Geometry: final body of the model. Coordinates: model frame, mm. A direction names the side the tool comes from. Round coordinates to 2 decimals unless told otherwise and drop trailing zeros. Write each loop counter-clockwise with the first axis right and the second up, starting at its lowest first coordinate (ties: lowest second). Pieces come first, ordered by that corner, then holes. Notation, with made-up numbers: (-40, 81.25) -> (7, 81.25) arc R22 ccw to (7, 88.25) -> close; hole circle Ø8 at (83, -39). An arc over 180 degrees is marked (long way). Use one line per item in the form item = value. Start each with the question number.
1. Cut plane C-C, the plane x = 6.5. Return the cut outline in (y, z), plus the area to 3 significant figures.
2. Line query: L1, parallel to X at y = 15.25, z = 154; L2, parallel to X at y = 3, z = 145.5; L3, parallel to Y at x = 11, z = 116.5. Output: solid intervals per line, ascending.
3. Pin query (flat end, axial travel): pin 1 Ø0.9 at (x, y) = (30.5, 14.5) entering from -Z; pin 2 Ø4 at (x, y) = (15, 4.5) entering from +Z; pin 3 Ø1.6 at (x, y) = (30.5, 12) entering from +Z; pin 4 Ø0.8 at (y, z) = (0.5, 49) entering from -X. Return the tip coordinate at first contact, or that it passes through.
4. Cut plane D-D, the plane z = 163.5. Return the cut outline in (x, y).
5. Cut plane A-A, the plane y = 6.5. Return the cut outline in (x, z).
6. Reachability of faces 1 (the face through (1.5, 11, 113)), 2 (the face through (0, 11, 113)) from +Z, -Z, +X, -X, +Y, -Y: full face, straight path, thin tool, end or side. Return the list, or none.
7. Draft query along X for faces 3 (the face through (16, 1.5, 116)), 4 (the face through (31.75, 11, 113)), 5 (the face through (30.25, 11, 113)), 6 (the face through (16, 0, 113)). Return one class per face: pulls with the +X half, pulls with the -X half, needs draft (parallel to the pull), parting line crosses it, or undercut.
8. Cut plane B-B, the plane z = 35. Return the cut outline in (x, y), plus the area to 3 significant figures.
```python
from build123d import *

# Parameters (mm, degrees)
BOSS_EXTRUDE1_DEPTH = 228.6
SKETCH2_W           = 19.05
SKETCH2_H           = 17.55
CUT_EXTRUDE1_DEPTH  = 232.579198116
CUT_EXTRUDE2_DEPTH  = 232.579198116


with BuildPart() as part:
    # Sketch1 → Boss-Extrude1 (new body)
    with BuildSketch(Plane.XY):
        with BuildLine():
            Line((30.25, 3.1), (30.25, 19.05))
            Line((30.25, 19.05), (31.75, 19.05))
            Line((31.75, 19.05), (31.75, 3.2))
            ThreePointArc((31.75, 3.2), (30.8127417, 0.9372583), (28.55, 0))
            Line((28.55, 0), (3.2, 0))
            ThreePointArc((3.2, 0), (0.9372583, 0.9372583), (0, 3.2))
            Line((0, 3.2), (0, 19.05))
            Line((0, 19.05), (1.5, 19.05))
            Line((1.5, 19.05), (1.5, 3.1))
            ThreePointArc((1.5, 3.1), (1.96862915, 1.96862915), (3.1, 1.5))
            Line((3.1, 1.5), (28.65, 1.5))
            ThreePointArc((28.65, 1.5), (29.78137085, 1.96862915), (30.25, 3.1))
        make_face()
    extrude(amount=BOSS_EXTRUDE1_DEPTH)

    # Sketch2 → Cut-Extrude1 (cut, through all)
    with BuildSketch(Plane(origin=(0, 0, 0), x_dir=(0, 0, -1), z_dir=(1, 0, 0))):
        with Locations((-9.525, 10.275)):
            Rectangle(SKETCH2_W, SKETCH2_H)
        with Locations((-219.075, 10.275)):
            Rectangle(SKETCH2_W, SKETCH2_H)
    extrude(amount=CUT_EXTRUDE1_DEPTH, mode=Mode.SUBTRACT)

    # Sketch3 → Cut-Extrude2 (cut, through all)
    with BuildSketch(Plane(origin=(0, 0, 0), x_dir=(1, 0, 0), z_dir=(0, 1, 0))):
        Polygon((22.821846385, -57.15), (8.928153615, -57.15), (8.928153615, -31.75), (9.428153615, -31.75), (9.428153615, -56.65), (22.321846385, -56.65), (22.321846385, -31.75), (22.821846385, -31.75), align=None)
    extrude(amount=CUT_EXTRUDE2_DEPTH, mode=Mode.SUBTRACT)


solid = part.part
```
Outcome:
q1.outline = (0, 0) -> (1.5, 0) -> (1.5, 228.6) -> (0, 228.6) -> close
q1.area = 343 mm^2
q2.L1 = 0 to 1.5, 30.25 to 31.75
q2.L2 = 0.01 to 1.5, 30.25 to 31.74
q2.L3 = 0 to 1.5
q3.pin_1 = 19.05
q3.pin_2 = through
q3.pin_3 = 209.55
q3.pin_4 = 0.98
q4.outline = (0, 3.2) arc R3.2 ccw to (3.2, 0) -> (28.55, 0) arc R3.2 ccw to (31.75, 3.2) -> (31.75, 19.05) -> (30.25, 19.05) -> (30.25, 3.1) arc R1.6 cw to (28.65, 1.5) -> (3.1, 1.5) arc R1.6 cw to (1.5, 3.1) -> (1.5, 19.05) -> (0, 19.05) -> close
q5.outline = (0, 19.05) -> (1.5, 19.05) -> (1.5, 209.55) -> (0, 209.55) -> close; (30.25, 19.05) -> (31.75, 19.05) -> (31.75, 209.55) -> (30.25, 209.55) -> close
q6.face_1 = +Z, -Z, +Y
q6.face_2 = +Z, -Z, -X, +Y, -Y
q7.face_3 = undercut
q7.face_4 = pulls with the +X half
q7.face_5 = undercut
q7.face_6 = needs draft
q8.outline = (0, 3.2) arc R3.2 ccw to (3.2, 0) -> (8.93, 0) -> (8.93, 1.5) -> (3.1, 1.5) arc R1.6 cw to (1.5, 3.1) -> (1.5, 19.05) -> (0, 19.05) -> close; (9.43, 0) -> (22.32, 0) -> (22.32, 1.5) -> (9.43, 1.5) -> close; (22.82, 0) -> (28.55, 0) arc R3.2 ccw to (31.75, 3.2) -> (31.75, 19.05) -> (30.25, 19.05) -> (30.25, 3.1) arc R1.6 cw to (28.65, 1.5) -> (22.82, 1.5) -> close
q8.area = 95.5 mm^2
